Geometry check sheet. Reference: the model listing, model coordinates, mm. A direction names the side the tool comes from. Round coordinates to 2 decimals unless told otherwise and drop trailing zeros. Loops run counter-clockwise (first coordinate to the right, second up) from the corner with the lowest first, then second, coordinate; pieces in that order, holes last.
```python
from build123d import *

# Parameters (mm, degrees)
SKETCH_1_R          = 100
SKETCH_1_R_2        = 30
EXTRUDE_1_DEPTH     = 40
SKETCH_2_R          = 100
SKETCH_2_R_2        = 90
CUT_EXTRUDE_1_DEPTH = 7.5


with BuildPart() as part:
    # 草图1 → 凸台-拉伸1 (new, symmetric)
    with BuildSketch(Plane.XY):
        Circle(SKETCH_1_R)
        Circle(SKETCH_1_R_2, mode=Mode.SUBTRACT)
    extrude(amount=EXTRUDE_1_DEPTH, both=True)

    # 草图2 → 切除-拉伸1 (cut, symmetric)
    with BuildSketch(Plane.XY.offset(20)):
        Circle(SKETCH_2_R)
        Circle(SKETCH_2_R_2, mode=Mode.SUBTRACT)
    cut_extrude_1 = extrude(amount=CUT_EXTRUDE_1_DEPTH, both=True, mode=Mode.SUBTRACT)

    # 镜向1: 切除-拉伸1 across plane
    add(cut_extrude_1.mirror(Plane.XY), mode=Mode.SUBTRACT)


solid = part.part
```
1) Mould release check, pull along Y, two halves, no side actions. Record for faces 1 (the face through (41.53, -79.845, -19.895)), 2 (the face through (-29.97, 1.32, -0.56)), 3 (the face through (-82, 38, -27.5)): +Y half, -Y half, draft (parallel to the pull), parting line (faces both ways), or undercut.
Report:
face 1: parting line
face 2: undercut
face 3: draft
2) Sectioned sample at C-C, the plane z = -22.5. Record the cut outline in (x, y).
Report:
outline: circle Ø180 at (0, 0); hole circle Ø60 at (0, 0)
3) Gauge pin test, flat ends, axial feed: pin 1 (3 mm diameter, centred on y = 73, z = -22.5, fed in from +X); pin 2 (1 mm diameter, centred on x = -34.5, z = 10, fed in from +Y); pin 3 (1 mm diameter, centred on y = 8, z = 25, fed in from +X). Record the tip position at first contact, or that the pin passes through.
Report:
pin 1: stops at x = 54.66
pin 2: stops at y = 94.04
pin 3: stops at x = 89.69
4) Sectioned sample at D-D, the plane y = 64. Record the cut outline in (x, z), then the cut area to 3 significant figures.
Report:
outline: (-76.84, -40) - (76.84, -40) - (76.84, -27.5) - (63.28, -27.5) - (63.28, -12.5) - (76.84, -12.5) - (76.84, 12.5) - (63.28, 12.5) - (63.28, 27.5) - (76.84, 27.5) - (76.84, 40) - (-76.84, 40) - (-76.84, 27.5) - (-63.28, 27.5) - (-63.28, 12.5) - (-76.84, 12.5) - (-76.84, -12.5) - (-63.28, -12.5) - (-63.28, -27.5) - (-76.84, -27.5) - close
area: 11,500 mm2
5) Scan lines: line 1 along Y through (x, z) = (0, -18.5); line 2 along X through (y, z) = (-13, -25.5); line 3 along X through (y, z) = (-10.5, 16). Record each from-to range of solid material in increasing order.
Report:
line 1: y = -90 to -30, 30 to 90
line 2: x = -89.06 to -27.04, 27.04 to 89.06
line 3: x = -89.39 to -28.1, 28.1 to 89.39
6) Sectioned sample at A-A, the plane y = 0. Record the cut outline in (x, z), then the cut area to 3 significant figures.
Report:
outline: (-100, -40) - (-30, -40) - (-30, 40) - (-100, 40) - (-100, 27.5) - (-90, 27.5) - (-90, 12.5) - (-100, 12.5) - (-100, -12.5) - (-90, -12.5) - (-90, -27.5) - (-100, -27.5) - close; (30, -40) - (100, -40) - (100, -27.5) - (90, -27.5) - (90, -12.5) - (100, -12.5) - (100, 12.5) - (90, 12.5) - (90, 27.5) - (100, 27.5) - (100, 40) - (30, 40) - close
area: 10,600 mm2
7) Access from +Z, -Z, +X, -X, +Y, -Y to the whole of each face (thin tool, end or side, straight path). Record for faces 4 (the face through (95.38, 30.04, 0.18)), 5 (the face through (-82, 38, -12.5)).
Report:
face 4: +Z, -Z
face 5: none
